For this review, use the dimensioned drawing (mm, ordinates from the lowest corner) and the shaded views. A direction names the side the tool comes from. Give positions to 0.01 mm unless a question says otherwise; leave off trailing zeros. Write each loop counter-clockwise with the first axis right and the second up, starting at its lowest first coordinate (ties: lowest second). Pieces come first, ordered by that corner, then holes. Notation, with made-up numbers: (54.5, 20.5) -> (73.5, 20.5) arc R28 ccw to (73.5, 56.5) -> close; hole circle Ø11 at (32.25, -36). An arc over 180 degrees is marked (long way). Return JSON: item names as keys, results as strings.
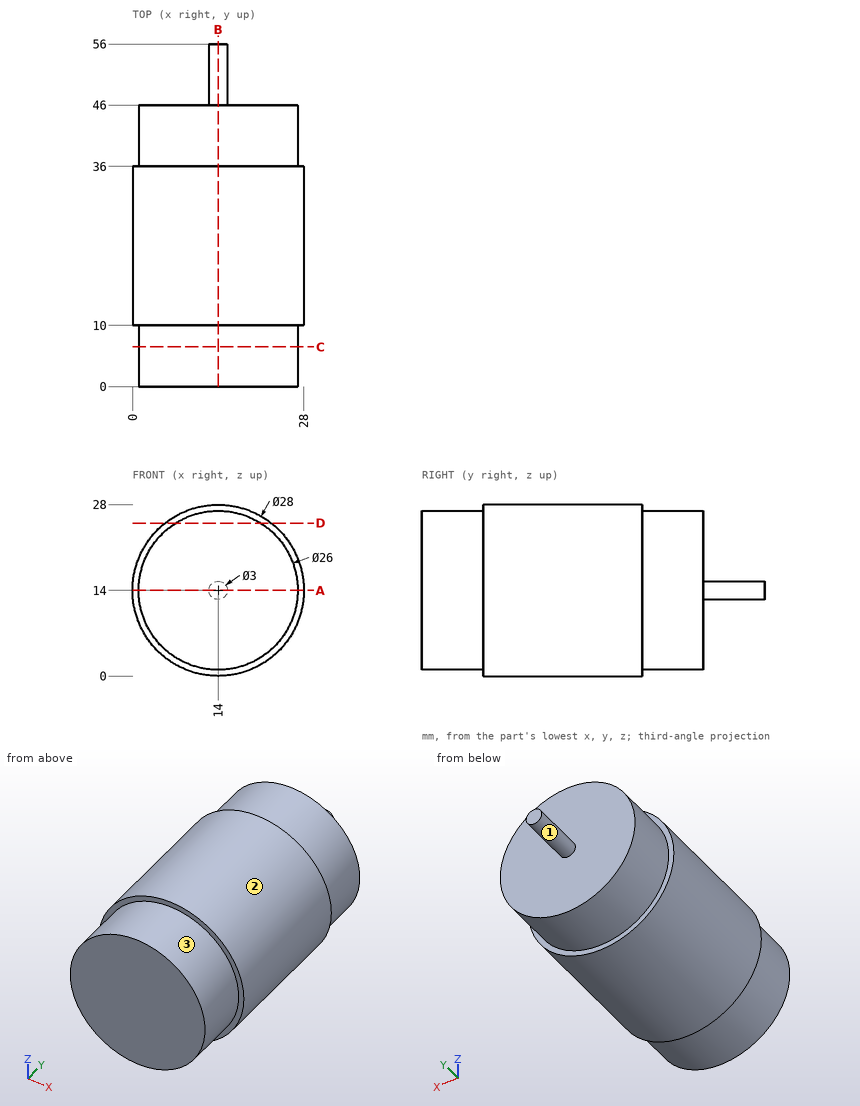
1. To check wall thickness, follow probe 1 along Y at (x, z) = (24, 6.5); probe 2 along X at (y, z) = (45, 14); probe 3 along X at (y, z) = (28.5, 2.75). State the ranges of each line that lie inside material, in increasing order.
Results found:
{"probe 1": "y = 0 to 46", "probe 2": "x = 1 to 27", "probe 3": "x = 5.67 to 22.33"}
2. Add section C-C, the plane y = 6.5. State the section outline as (x, z) points, plus the area to 3 significant figures.
Results found:
{"outline": "circle Ø26 at (14, 14)", "area": "531 mm²"}
3. Add section D-D, the plane z = 25. State the section outline as (x, y) points, plus the area to 3 significant figures.
Results found:
{"outline": "(5.34, 10) -> (7.07, 10) -> (7.07, 0) -> (20.93, 0) -> (20.93, 10) -> (22.66, 10) -> (22.66, 36) -> (20.93, 36) -> (20.93, 46) -> (7.07, 46) -> (7.07, 36) -> (5.34, 36) -> close", "area": "727 mm²"}
4. For the marked faces 1, 2 and 3, list the 3-axis set-ups (+Z, -Z, +X, -X, +Y, -Y) from which the entire face can be reached by the end or side of a thin tool; tool diameter is ignored.
Results found:
{"face 1": "+Y", "face 2": "+Y, -Y", "face 3": "-Y"}
5. Add section B-B, the plane x = 14. State the section outline as (y, z) points, plus the area to 3 significant figures.
Results found:
{"outline": "(0, 1) -> (10, 1) -> (10, 0) -> (36, 0) -> (36, 1) -> (46, 1) -> (46, 12.5) -> (56, 12.5) -> (56, 15.5) -> (46, 15.5) -> (46, 27) -> (36, 27) -> (36, 28) -> (10, 28) -> (10, 27) -> (0, 27) -> close", "area": "1,280 mm²"}
6. Add section A-A, the plane z = 14. State the section outline as (x, y) points, plus the area to 3 significant figures.
Results found:
{"outline": "(0, 10) -> (1, 10) -> (1, 0) -> (27, 0) -> (27, 10) -> (28, 10) -> (28, 36) -> (27, 36) -> (27, 46) -> (15.5, 46) -> (15.5, 56) -> (12.5, 56) -> (12.5, 46) -> (1, 46) -> (1, 36) -> (0, 36) -> close", "area": "1,280 mm²"}
7. For pin 1 (2 mm diameter, centred on y = 16, z = 24.5, fed in from -X); pin 2 (4 mm diameter, centred on y = 28, z = 19, fed in from -X); pin 3 (14 mm diameter, centred on x = 16.5, z = 12.5, fed in from -Y); pin 4 (1 mm diameter, centred on y = 27.5, z = 23, fed in from +X), all flat-tipped, find the tip position at first contact; note any pin that passes through.
Results found:
{"pin 1": "stops at x = 3.72", "pin 2": "stops at x = 0.33", "pin 3": "stops at y = 0", "pin 4": "stops at x = 25.12"}
